Input: part model. Units: mm. Frame: model coordinates. Face numbers are marked on the shaded views. A direction names the side the tool comes from. Give positions to 0.01 mm unless a question says otherwise; leave off trailing zeros. Loops run counter-clockwise (first coordinate to the right, second up) from the corner with the lowest first, then second, coordinate; pieces in that order, holes last. Notation, with made-up numbers: M 39.5,1.5 L 56.5,1.5 A32 ccw 56.5,34.5 Z; hole C 6.5,38.5 d10. An arc over 180 degrees is marked long. Answer as a JSON object with one key per item and string values. Group by question number.
1) First-contact query: P1, Ø2, axis at x = 8, y = 4, coming from the +Z side; P2, Ø6, axis at x = 3.5, z = 12.5, coming from the -Y side; P3, Ø1.5, axis at y = 7.5, z = 7.5, coming from the +X side. Flat tips, straight axial feed; report the tip coordinate or a pass-through.
2) Access query for the marked faces 1, 2 and 3. Directions: +Z, -Z, +X, -X, +Y, -Y. A direction counts if a zero-diameter tool reaches every point of the face in a straight line with its end or side. Return the directions, or none.
3) Section query A-A on y = 10. Return loops of the section in (x, z), plus the area to 3 significant figures.
4) Section query D-D on x = -4.5. Return loops of the section in (y, z), plus the area to 3 significant figures.
5) Ray query, L1, parallel to Z at x = -5.75, y = 13.75; L2, parallel to X at y = 7, z = 7; L3, parallel to Y at x = -0.5, z = -10. Return the intervals inside material, ascending.
6) Section query B-B on x = 0. Return loops of the section in (y, z).
7) Section query C-C on z = -12. Return loops of the section in (x, y), plus the area to 3 significant figures.
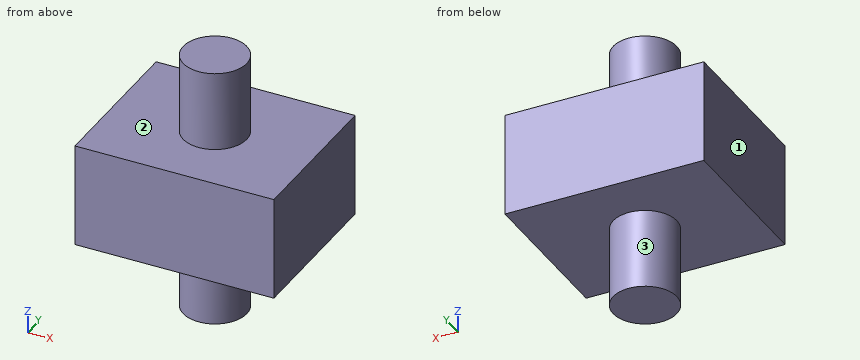
from build123d import *

# Parameters (mm, degrees)
SKETCH1_W           = 25
SKETCH1_H           = 13
BOSS_EXTRUDE1_DEPTH = 20
SKETCH2_R           = 4
BOSS_EXTRUDE2_DEPTH = 10


with BuildPart() as part:
    # Sketch1 → Boss-Extrude1 (new body)
    with BuildSketch(Plane(origin=(0, 0, 0), x_dir=(1, 0, 0), z_dir=(0, 1, 0))):
        Rectangle(SKETCH1_W, SKETCH1_H)
    extrude(amount=BOSS_EXTRUDE1_DEPTH)

    # Sketch2 → Boss-Extrude2 (add)
    with BuildSketch(Plane.XY.offset(6.5)):
        with Locations((0, 10)):
            Circle(SKETCH2_R)
    boss_extrude2 = extrude(amount=BOSS_EXTRUDE2_DEPTH)

    # Mirror1: Boss-Extrude2 across plane
    add(boss_extrude2.mirror(Plane.XY))


solid = part.part
Output:
{
 "1": {"P1": "stops at z = 6.5", "P2": "stops at y = 6.03", "P3": "stops at x = 3.6"},
 "2": {"face 1": "+Z, -Z, -X, +Y, -Y", "face 2": "+Z", "face 3": "-Z"},
 "3": {"outline": "M -12.5,-6.5 L -4,-6.5 L -4,-16.5 L 4,-16.5 L 4,-6.5 L 12.5,-6.5 L 12.5,6.5 L 4,6.5 L 4,16.5 L -4,16.5 L -4,6.5 L -12.5,6.5 Z", "area": "485 mm^2"},
 "4": {"outline": "M 0,-6.5 L 20,-6.5 L 20,6.5 L 0,6.5 Z", "area": "260 mm^2"},
 "5": {"L1": "z = -6.5 to 6.5", "L2": "x = -2.65 to 2.65", "L3": "y = 6.03 to 13.97"},
 "6": {"outline": "M 0,-6.5 L 6,-6.5 L 6,-16.5 L 14,-16.5 L 14,-6.5 L 20,-6.5 L 20,6.5 L 14,6.5 L 14,16.5 L 6,16.5 L 6,6.5 L 0,6.5 Z"},
 "7": {"outline": "C 0,10 d8", "area": "50.3 mm^2"}
}
